```python
from build123d import *

# Parameters (mm, degrees)
EXTRUDE_1_DEPTH     = 6.2
SKETCH_3_R          = 5
EXTRUDE_3_DEPTH     = 45
SKETCH_5_OUTSIDE_W  = 375.758
SKETCH_5_OUTSIDE_H  = 378.234
SKETCH_5_OUTSIDE_R  = 8
CUT_EXTRUDE_2_DEPTH = 100
CUT_EXTRUDE_2_DRAFT = -60
CHAMFER_1_SIZE      = 1.25
SKETCH_2_OUTSIDE_W  = 29.346
SKETCH_2_OUTSIDE_H  = 31.822
SKETCH_2_OUTSIDE_R  = 7.2
CUT_EXTRUDE_1_DEPTH = 0.413333333
FILLET_1_R          = 0.1


with BuildPart() as part:
    # 草图1 → 凸台-拉伸1 (new body)
    with BuildSketch(Plane.XY):
        Polygon((0, 9.237604307), (-8, 4.618802154), (-8, -4.618802154), (0, -9.237604307), (8, -4.618802154), (8, 4.618802154), align=None)
    extrude(amount=EXTRUDE_1_DEPTH)

    # 草图3 → 凸台-拉伸3 (add)
    with BuildSketch(Plane.XY):
        Circle(SKETCH_3_R)
    extrude(amount=-EXTRUDE_3_DEPTH)


with BuildPart() as cut_extrude_2_tool:
    # 草图5 outside → 切除-拉伸2 (with draft: the straight prism first)
    with BuildSketch(Plane.XY.offset(6.2)):
        Rectangle(SKETCH_5_OUTSIDE_W, SKETCH_5_OUTSIDE_H)
        Circle(SKETCH_5_OUTSIDE_R, mode=Mode.SUBTRACT)
    extrude(amount=-CUT_EXTRUDE_2_DEPTH)
    # 切除-拉伸2: the draft: its side faces are tilted about the plane it starts from
    cut_extrude_2_sides = [cut_extrude_2_tool.faces().sort_by_distance(p)[0] for p in [
        (0, -189.117, -43.8),
        (187.879, 0, -43.8),
        (0, 189.117, -43.8),
        (-187.879, 0, -43.8),
        (-8, 0, -43.8),
    ]]
    draft(cut_extrude_2_sides, Plane.XY.offset(6.2), CUT_EXTRUDE_2_DRAFT)


with BuildPart() as part_1:
    add(part.part)

    # 切除-拉伸2: cut by cut_extrude_2_tool
    add(cut_extrude_2_tool.part, mode=Mode.SUBTRACT)

    # 倒角1
    chamfer_1_edges = [part_1.edges().sort_by_distance(p)[0] for p in [
        (-5, 0, -45),
    ]]
    chamfer(chamfer_1_edges, length=CHAMFER_1_SIZE)

    # 草图2 outside → 切除-拉伸1 (cut)
    with BuildSketch(Plane.XY):
        Rectangle(SKETCH_2_OUTSIDE_W, SKETCH_2_OUTSIDE_H)
        Circle(SKETCH_2_OUTSIDE_R, mode=Mode.SUBTRACT)
    extrude(amount=CUT_EXTRUDE_1_DEPTH, mode=Mode.SUBTRACT)

    # 圆角1
    fillet_1_edges = [part_1.edges().sort_by_distance(p)[0] for p in [
        (-5, 0, 0),
    ]]
    fillet(fillet_1_edges, radius=FILLET_1_R)


solid = part_1.part
```
Verification items for the finished model (mm, model axes). A direction names the side the tool comes from. Give positions to 0.01 mm unless a question says otherwise; leave off trailing zeros. Order: outer loops, then holes, each group sorted by start corner. A loop starts at its lowest first (then second) coordinate and runs counter-clockwise, first axis right, second up. Notation, with made-up numbers: (60.5, 76) -> (113.5, 76) arc R19 ccw to (113.5, 99) -> close; hole circle Ø11 at (82.5, 72.5). An arc over 180 degrees is marked (long way). Use a Markdown table: item, result.
1) Material ranges on probe 1 along Y at (x, z) = (3, -20); probe 2 along Z at (x, y) = (-5.25, 4.25); probe 3 along Z at (x, y) = (5.75, 5.25), recorded low to high.
Results:
| item | result |
|---|---|
| probe 1 | -4 to 4 |
| probe 2 | 0 to 6.2 |
| probe 3 | 0.41 to 6.2 |
2) Tool access check on faces 1 (the conical face through (7.17, -4.17, 6.03)), 2 (the cylindrical face through (6.87, 2.16, 0.2)). Record the directions out of +Z, -Z, +X, -X, +Y, -Y that give a thin tool (end or side, any length) a straight path to the whole face; none if there is none.
Results:
| item | result |
|---|---|
| face 1 | +Z, +X, -Y |
| face 2 | -Z |
3) Section check A-A, the plane z = -30.5. Record the boundary of the cut face in (x, y), then the cut area to 3 significant figures.
Results:
| item | result |
|---|---|
| outline | circle Ø10 at (0, 0) |
| area | 78.5 mm² |
4) Depth check by flat-ended pin: pin 1 Ø1 at (x, z) = (-4, -20.5) entering from -Y; pin 2 Ø2 at (x, y) = (-0.5, 7) entering from -Z; pin 3 Ø4 at (y, z) = (-0.5, -37) entering from +X. Enter the tip coordinate at first touch or a pass-through.
Results:
| item | result |
|---|---|
| pin 1 | y = -3.57 |
| pin 2 | z = 0 |
| pin 3 | x = 5 |
